Study the drawing (mm; zero at the part's minimum x, y, z) and answer. Give positions to 0.01 mm unless a question says otherwise; leave off trailing zeros. Write each loop counter-clockwise with the first axis right and the second up, starting at its lowest first coordinate (ties: lowest second). Pieces come first, ordered by that corner, then holes.
1) Given pin 1 Ø5.5 at (x, y) = (8, 10) entering from -Z; pin 2 Ø7 at (x, y) = (7.5, 10.5) entering from -Z, each flat-ended and moving along its own axis, determine where each tip first touches the part or whether it passes through.
2) Find section B-B (x = 8). Determine the outline of the cut face in (y, z), plus the area to 3 significant figures.
3) Find section C-C (z = 2). Determine the outline of the cut face in (x, y), plus the area to 3 significant figures.
4) Find section A-A (y = 10). Determine the outline of the cut face in (x, z).
5) Straight lines are drawn through the part: probe 1 along Y at (x, z) = (8, 5.5); probe 2 along Y at (x, z) = (8, 3.95); probe 3 along Z at (x, y) = (4, 12). For each, find the intervals that lie inside material, in ascending order.
6) Find section D-D (z = 8). Determine the outline of the cut face in (x, y).
7) Determine the mould class of the marked faces 1, 2 and 3 for opening direction Y: pulls with the +Y half, pulls with the -Y half, needs draft (parallel to the pull), parting line crosses it, or undercut.
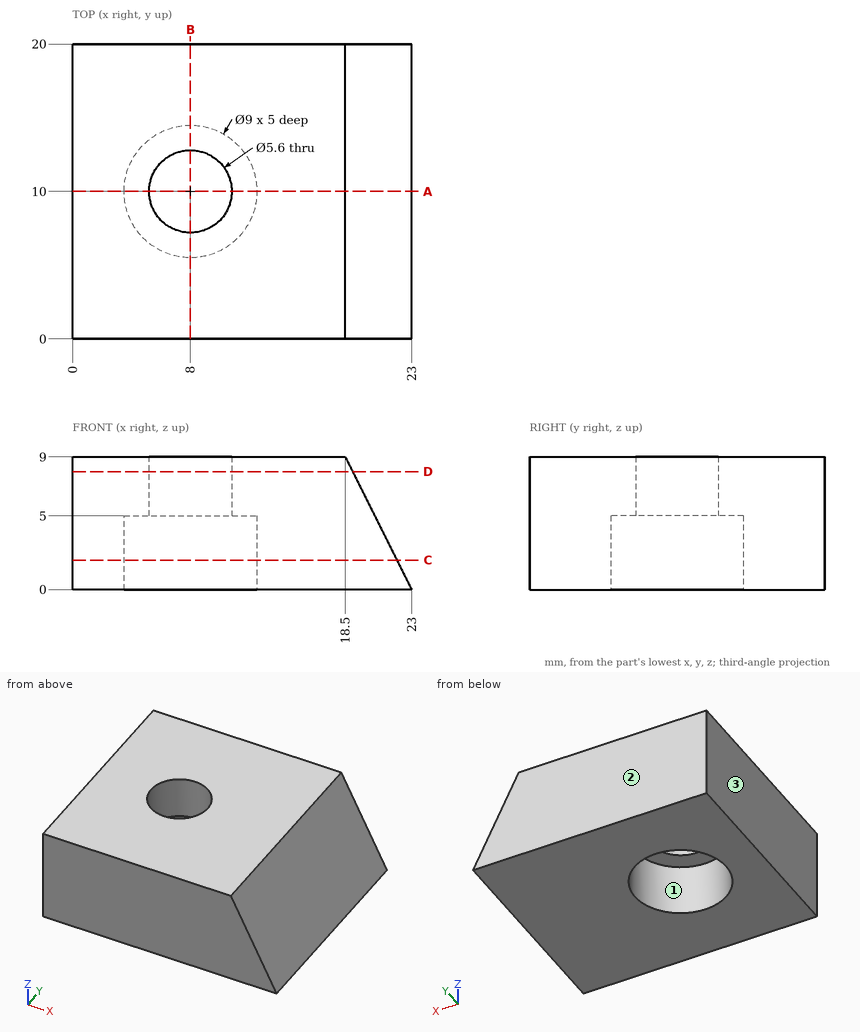
Results:
1. pin 1: passes through
1. pin 2: stops at z = 5
2. outline: (0, 0) - (5.5, 0) - (5.5, 5) - (7.2, 5) - (7.2, 9) - (0, 9) - close; (12.8, 5) - (14.5, 5) - (14.5, 0) - (20, 0) - (20, 9) - (12.8, 9) - close
2. area: 113 mm2
3. outline: (0, 0) - (22, 0) - (22, 20) - (0, 20) - close; hole circle Ø9 at (8, 10)
3. area: 376 mm2
4. outline: (0, 0) - (3.5, 0) - (3.5, 5) - (5.2, 5) - (5.2, 9) - (0, 9) - close; (10.8, 5) - (12.5, 5) - (12.5, 0) - (23, 0) - (18.5, 9) - (10.8, 9) - close
5. probe 1: y = 0 to 7.2, 12.8 to 20
5. probe 2: y = 0 to 5.5, 14.5 to 20
5. probe 3: z = 5 to 9
6. outline: (0, 0) - (19, 0) - (19, 20) - (0, 20) - close; hole circle Ø5.6 at (8, 10)
7. face 1: undercut
7. face 2: pulls with the +Y half
7. face 3: needs draft
